```python
from build123d import *

# Parameters (mm, degrees)
SKETCH_1_R          = 450
EXTRUDE_1_DEPTH     = 12
SKETCH_2_R          = 375
EXTRUDE_2_DEPTH     = 13
SKETCH_3_R          = 20
CUT_EXTRUDE_2_DEPTH = 314
SKETCH_4_R          = 350
CUT_EXTRUDE_3_DEPTH = 314


with BuildPart() as part:
    # 草图1 → 凸台-拉伸1 (new body)
    with BuildSketch(Plane.XY):
        Circle(SKETCH_1_R)
    extrude(amount=EXTRUDE_1_DEPTH)

    # 草图2 → 凸台-拉伸2 (add)
    with BuildSketch(Plane.XY.offset(12)):
        with Locations(Location((0, 0, 0), (0, 0, 180))):
            Circle(SKETCH_2_R)
    extrude(amount=EXTRUDE_2_DEPTH)

    # 草图3 → 切除-拉伸2 (cut)
    with BuildSketch(Plane(origin=(0, 0, 0), x_dir=(-1, 0, 0), z_dir=(0, 0, -1))):
        with Locations((0, 410)):
            Circle(SKETCH_3_R)
        with Locations((106.115808492, 396.029588779)):
            Circle(SKETCH_3_R)
        with Locations((205, 355.070415552)):
            Circle(SKETCH_3_R)
        with Locations((289.913780286, 289.913780286)):
            Circle(SKETCH_3_R)
        with Locations((355.070415552, 205)):
            Circle(SKETCH_3_R)
        with Locations((396.029588779, 106.115808492)):
            Circle(SKETCH_3_R)
        with Locations((410, 0)):
            Circle(SKETCH_3_R)
        with Locations((396.029588779, -106.115808492)):
            Circle(SKETCH_3_R)
        with Locations((355.070415552, -205)):
            Circle(SKETCH_3_R)
        with Locations((289.913780286, -289.913780286)):
            Circle(SKETCH_3_R)
        with Locations((205, -355.070415552)):
            Circle(SKETCH_3_R)
        with Locations((106.115808492, -396.029588779)):
            Circle(SKETCH_3_R)
        with Locations((0, -410)):
            Circle(SKETCH_3_R)
        with Locations((-106.115808492, -396.029588779)):
            Circle(SKETCH_3_R)
        with Locations((-205, -355.070415552)):
            Circle(SKETCH_3_R)
        with Locations((-289.913780286, -289.913780286)):
            Circle(SKETCH_3_R)
        with Locations((-355.070415552, -205)):
            Circle(SKETCH_3_R)
        with Locations((-396.029588779, -106.115808492)):
            Circle(SKETCH_3_R)
        with Locations((-410, 0)):
            Circle(SKETCH_3_R)
        with Locations((-396.029588779, 106.115808492)):
            Circle(SKETCH_3_R)
        with Locations((-355.070415552, 205)):
            Circle(SKETCH_3_R)
        with Locations((-289.913780286, 289.913780286)):
            Circle(SKETCH_3_R)
        with Locations((-205, 355.070415552)):
            Circle(SKETCH_3_R)
        with Locations((-106.115808492, 396.029588779)):
            Circle(SKETCH_3_R)
    extrude(amount=-CUT_EXTRUDE_2_DEPTH, mode=Mode.SUBTRACT)

    # 草图4 → 切除-拉伸3 (cut)
    with BuildSketch(Plane.XY.offset(25)):
        Circle(SKETCH_4_R)
    extrude(amount=-CUT_EXTRUDE_3_DEPTH, mode=Mode.SUBTRACT)


solid = part.part
```
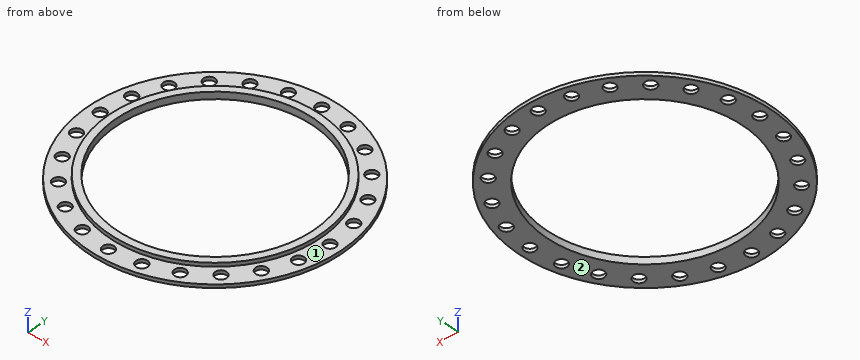
The model under review builds one solid part; all positions refer to its coordinate system, in mm. Face numbers are marked on the shaded views. A direction names the side the tool comes from. Round coordinates to 2 decimals unless told otherwise and drop trailing zeros. Order: outer loops, then holes, each group sorted by start corner. A loop starts at its lowest first (then second) coordinate and runs counter-clockwise, first axis right, second up. Notation, with made-up numbers: (50.25, 69.5) - (89.25, 69.5) arc R15 ccw to (89.25, 74.5) - close; hole circle Ø1 at (41, -23). An arc over 180 degrees is marked (long way). Answer in a Markdown table with one row per item.
(1) Machinability: for the marked faces 1 and 2, which of the approach directions +Z, -Z, +X, -X, +Y, -Y give a long, thin tool a straight path to every point of the face, cutting with its end or side? Answer none if there is none.
Result set:
| item | result |
|---|---|
| face 1 | +Z |
| face 2 | -Z, +X, -X, +Y, -Y |
(2) Take a section at A-A on x = 0. Write out the cut boundary in (y, z).
Result set:
| item | result |
|---|---|
| outline | (-450, 0) - (-430, 0) - (-430, 12) - (-450, 12) - close; (-390, 0) - (-350, 0) - (-350, 25) - (-375, 25) - (-375, 12) - (-390, 12) - close; (350, 0) - (390, 0) - (390, 12) - (375, 12) - (375, 25) - (350, 25) - close; (430, 0) - (450, 0) - (450, 12) - (430, 12) - close |
(3) Clearance check with flat-ended pins moving along their axes: P1, Ø6, axis at y = -268.5, z = 10, coming from the -X side; P2, Ø4, axis at x = -271, z = 11.5, coming from the +Y side; P3, Ø5, axis at x = 339.5, z = 5, coming from the +Y side. State where each tip first meets the part, or that it passes through.
Result set:
| item | result |
|---|---|
| P1 | stops at x = -363.33 |
| P2 | stops at y = 360.75 |
| P3 | stops at y = 298.21 |
(4) For line 1 (Y direction, x = 0, z = 3.25); line 2 (X direction, y = 7.5, z = 7); line 3 (Y direction, x = 124.5, z = 9.5), list the stretches that pass through material, from the lowest coordinate up. Write a range as from..to.
Result set:
| item | result |
|---|---|
| line 1 | y = -450..-430, -390..-350, 350..390, 430..450 |
| line 2 | x = -449.94..-428.54, -391.46..-349.92, 349.92..391.46, 428.54..449.94 |
| line 3 | y = -432.43..-403.9, -388.15..-327.11, 327.11..388.15, 403.9..432.43 |
(5) Take a section at C-C on z = 17.5. Write out the cut boundary in (x, y), plus the area to 3 significant figures.
Result set:
| item | result |
|---|---|
| outline | circle Ø750 at (0, 0); hole circle Ø700 at (0, 0) |
| area | 56,900 mm2 |
